Geometry check sheet. Reference: the model listing, model coordinates, mm. Face numbers are marked on the shaded views. A direction names the side the tool comes from. Coordinates: 2 decimals unless noted, no trailing zeros. Loops run counter-clockwise (first coordinate to the right, second up) from the corner with the lowest first, then second, coordinate; pieces in that order, holes last. Notation, with made-up numbers: (75, 34.5) - (111, 34.5) arc R26 ccw to (111, 61.5) - close; hole circle Ø8 at (80.5, -6.75). An arc over 180 degrees is marked (long way). Write each question's results on one line, items separated by ' | '. Start each with the question number.
(1) Access from +Z, -Z, +X, -X, +Y, -Y to the whole of each face (thin tool, end or side, straight path). Record for the marked faces 1 and 2.
(2) Sectioned sample at C-C (z = 16). Enter the section's corners in (x, y), plus the area to 3 significant figures.
(3) Sectioned sample at D-D (x = -14). Enter the section's corners in (y, z).
(4) Go/stop test with flat-tipped pins: pin 1 Ø1.5 at (y, z) = (-1, 80) entering from +X; pin 2 Ø6.5 at (x, y) = (-17.68, -17.68) entering from +Z; pin 3 Ø1 at (y, z) = (3, 40.5) entering from -X. Record where each tip stops, or that it passes through.
(5) Sectioned sample at A-A (x = 0). Enter the section's corners in (y, z), plus the area to 3 significant figures.
(6) Material ranges on probe 1 along Z at (x, y) = (-14, -7.5); probe 2 along Z at (x, y) = (4.5, 10); probe 3 along Y at (x, z) = (0, 54.5), recorded low to high.
from build123d import *

# Parameters (mm, degrees)
SKETCH1_W           = 45
SKETCH1_H           = 45
SKETCH1_R           = 2.5
BOSS_EXTRUDE1_DEPTH = 10
SKETCH2_R           = 11
BOSS_EXTRUDE2_DEPTH = 105
CHAMFER1_SIZE       = 1
CUT_EXTRUDE1_START  = -5
SKETCH3_R           = 12.248377089
SKETCH3_R_2         = 10
CUT_EXTRUDE1_DEPTH  = 1.2


with BuildPart() as part:
    # Sketch1 → Boss-Extrude1 (new body)
    with BuildSketch(Plane.XY):
        Rectangle(SKETCH1_W, SKETCH1_H)
        with Locations((17.67766953, 17.67766953)):
            Circle(SKETCH1_R, mode=Mode.SUBTRACT)
        with Locations((17.67766953, -17.67766953)):
            Circle(SKETCH1_R, mode=Mode.SUBTRACT)
        with Locations((-17.67766953, -17.67766953)):
            Circle(SKETCH1_R, mode=Mode.SUBTRACT)
        with Locations((-17.67766953, 17.67766953)):
            Circle(SKETCH1_R, mode=Mode.SUBTRACT)
    extrude(amount=BOSS_EXTRUDE1_DEPTH)

    # Sketch2 → Boss-Extrude2 (add)
    with BuildSketch(Plane.XY.offset(10)):
        Circle(SKETCH2_R)
    extrude(amount=BOSS_EXTRUDE2_DEPTH)

    # Chamfer1
    chamfer1_edges = [part.edges().sort_by_distance(p)[0] for p in [
        (-11, 0, 115),
    ]]
    chamfer(chamfer1_edges, length=CHAMFER1_SIZE)

    # Sketch3 → Cut-Extrude1 (cut)
    with BuildSketch(Plane.XY.offset(115).offset(CUT_EXTRUDE1_START)):
        Circle(SKETCH3_R)
        Circle(SKETCH3_R_2, mode=Mode.SUBTRACT)
    extrude(amount=-CUT_EXTRUDE1_DEPTH, mode=Mode.SUBTRACT)


solid = part.part
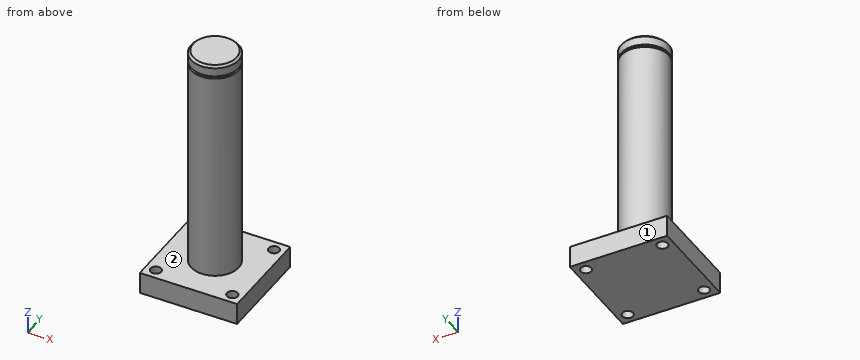
Outcome:
1) face 1: +Z, -Z, +X, -X, +Y | face 2: +Z
2) outline: circle Ø22 at (0, 0) | area: 380 mm2
3) outline: (-22.5, 0) - (22.5, 0) - (22.5, 10) - (-22.5, 10) - close
4) pin 1: stops at x = 11 | pin 2: stops at z = 10 | pin 3: stops at x = -10.71
5) outline: (-22.5, 0) - (22.5, 0) - (22.5, 10) - (11, 10) - (11, 108.8) - (10, 108.8) - (10, 110) - (11, 110) - (11, 114) - (10, 115) - (-10, 115) - (-11, 114) - (-11, 110) - (-10, 110) - (-10, 108.8) - (-11, 108.8) - (-11, 10) - (-22.5, 10) - close | area: 2,760 mm2
6) probe 1: z = 0 to 10 | probe 2: z = 0 to 108.8, 110 to 114.03 | probe 3: y = -11 to 11
